Design review of the part built by this model. Coordinates are the model's own, in mm. Face numbers are marked on the shaded views. A direction names the side the tool comes from. Coordinates: 2 decimals unless noted, no trailing zeros. Loops run counter-clockwise (first coordinate to the right, second up) from the corner with the lowest first, then second, coordinate; pieces in that order, holes last. Notation, with made-up numbers: M -3,-15.5 L 22,-15.5 A21 cw 22,2.5 Z; hole C -22.5,87 d3. An arc over 180 degrees is marked long. Write item = value, one per line. Start each with the question number.
from build123d import *

# Parameters (mm, degrees)
EXTRUDE_1_DEPTH       = 15
EXTRUDE_2_DEPTH       = 8
CUT_EXTRUDE_1_DEPTH   = 12
CUT_EXTRUDE_2_DEPTH   = 8
SKETCH_5_R            = 0.5
CUT_EXTRUDE_3_DEPTH   = 317.640652423
SKETCH_6_R            = 2.75
CUT_EXTRUDE_4_DEPTH   = 317.640652423
HOLE_WIZARD_3_0_3_1_D = 6.5
HOLE_WIZARD_M3_1_D    = 2.5


with BuildPart() as part:
    # 草图1 → 凸台-拉伸1 (new body)
    with BuildSketch(Plane.XY):
        with BuildLine():
            Line((154.501486248, 74.365814355), (160.177770707, 76.310041404))
            ThreePointArc((160.177770707, 76.310041404), (169.160526734, 140.718106761), (226.383321785, 171.615364171))
            Line((226.383321785, 171.615364171), (225.315728088, 174.727294301))
            Line((225.315728088, 174.727294301), (234.77220836, 177.96630476))
            Line((234.77220836, 177.96630476), (231.998602564, 186.064008926))
            Line((231.998602564, 186.064008926), (230.57080221, 190.225905867))
            Line((230.57080221, 190.225905867), (233.408459215, 191.199406109))
            Line((233.408459215, 191.199406109), (233.213759167, 191.76693751))
            Line((233.213759167, 191.76693751), (240.591667381, 194.298038138))
            Line((240.591667381, 194.298038138), (240.786367429, 193.730506737))
            Line((240.786367429, 193.730506737), (243.624024434, 194.704006979))
            Line((243.624024434, 194.704006979), (241.482323903, 200.94685239))
            Line((241.482323903, 200.94685239), (129.111106493, 162.396242824))
            Line((129.111106493, 162.396242824), (132.680607379, 151.991500471))
            Line((132.680607379, 151.991500471), (154.501486248, 74.365814355))
        make_face()
    extrude(amount=EXTRUDE_1_DEPTH)

    # 草图2 → 凸台-拉伸2 (add)
    with BuildSketch(Plane(origin=(0, 0, 0), x_dir=(-1, 0, 0), z_dir=(0, 0, -1))):
        Polygon((-174.908927271, 177.441379972), (-194.997272817, 184.33298428), (-193.224414699, 175.267097261), (-181.873786677, 171.373096295), align=None)
    extrude(amount=EXTRUDE_2_DEPTH)

    # 草图3 → 切除-拉伸1 (cut)
    with BuildSketch(Plane.XY.offset(15)):
        with BuildLine():
            Line((148.33581351, 109.973924886), (137.488957816, 148.560574876))
            ThreePointArc((137.488957816, 148.560574876), (137.68708728, 150.700674405), (139.265834382, 152.159042969))
            Line((139.265834382, 152.159042969), (212.284799547, 181.275892717))
            ThreePointArc((212.284799547, 181.275892717), (214.647795853, 181.215617846), (216.233642795, 179.462770427))
            Line((216.233642795, 179.462770427), (217.297595906, 176.361452247))
            ThreePointArc((217.297595906, 176.361452247), (217.048600661, 173.871762608), (214.998888251, 172.436760111))
            ThreePointArc((214.998888251, 172.436760111), (175.157111586, 151.143900213), (155.117593814, 110.657226135))
            ThreePointArc((155.117593814, 110.657226135), (154.455434588, 109.182984766), (153.12452466, 108.266185323))
            Line((153.12452466, 108.266185323), (152.197376559, 107.948113442))
            ThreePointArc((152.197376559, 107.948113442), (149.830188599, 108.129149559), (148.33581351, 109.973924886))
        make_face()
    extrude(amount=-CUT_EXTRUDE_1_DEPTH, mode=Mode.SUBTRACT)

    # 草图4 → 切除-拉伸2 (cut)
    with BuildSketch(Plane.XY.offset(15)):
        Polygon((234.77220836, 177.96630476), (225.315728088, 174.727294301), (222.53974588, 182.819008121), (231.998602564, 186.064008926), align=None)
    extrude(amount=-CUT_EXTRUDE_2_DEPTH, mode=Mode.SUBTRACT)

    # 草图5 → 切除-拉伸3 (cut, through all)
    with BuildSketch(Plane.XY.offset(15)):
        with Locations((228.656571223, 180.394154027)):
            Circle(SKETCH_5_R)
    extrude(amount=-CUT_EXTRUDE_3_DEPTH, mode=Mode.SUBTRACT)

    # 草图6 → 切除-拉伸4 (cut, through all)
    with BuildSketch(Plane.XY.offset(15)):
        with Locations((138.625192324, 159.316929458)):
            Circle(SKETCH_6_R)
        with Locations((222.809016814, 188.197436624)):
            Circle(SKETCH_6_R)
    extrude(amount=-CUT_EXTRUDE_4_DEPTH, mode=Mode.SUBTRACT)

    # Ø3.0 (3) 直径孔1 (through all)
    with Locations(Plane(origin=(-34.303459783, 99.991195485, 0), x_dir=(-0.9458856684292948, -0.32450008052397505, 0), z_dir=(0.32450008052397505, -0.9458856684292948, 0))):
        with Locations((-286.72193914, -5)):
            Hole(HOLE_WIZARD_3_0_3_1_D / 2)

    # M3 螺纹孔1 (through all)
    with Locations(Plane.XY.offset(7)):
        with Locations((228.656571223, 180.394154027)):
            Hole(HOLE_WIZARD_M3_1_D / 2)


solid = part.part
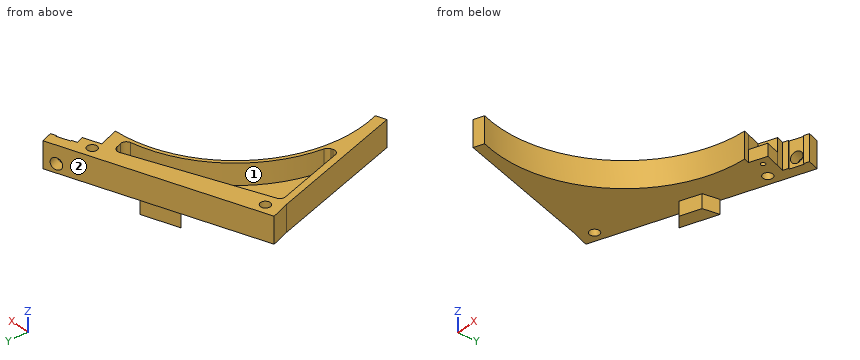
Q1. To check wall thickness, follow line 1 (Y direction, x = 182.5, z = 12.5); line 2 (X direction, y = 134.5, z = 10.5); line 3 (Z direction, x = 149, y = 133). State the ranges of each line that lie inside material, in increasing order. Write a range as from..to.
Q2. Add section B-B on y = 125. State the section outline as (x, z) points, plus the area to 3 significant figures.
Q3. Add section D-D on z = -3. State the section outline as (x, y) points, plus the area to 3 significant figures.
Q4. Add section C-C on x = 205. State the section outline as (y, z) points.
Q5. Clearance check with flat-ended pins moving along their axes: P1, Ø12, axis at x = 204, z = -5, coming from the +Y side; P2, Ø4, axis at y = 152, z = 6, coming from the -X side; P3, Ø2, axis at x = 147.5, z = 11, coming from the +Y side. State where each tip first meets the part, or that it passes through.
Q6. For the marked faces 1 and 2, list the 3-axis set-ups (+Z, -Z, +X, -X, +Y, -Y) from which the entire face can be reached by the end or side of a thin tool; tool diameter is ignored.
Q7. Add section A-A on z = 10.5. State the section outline as (x, y) points.
Values follow:
q1.line_1 = 155.2..157.77, 169.4..180.71
q1.line_2 = 137.6..141.44, 163.02..165.29
q1.line_3 = 0..3
q2.outline = M 140.27,0 L 160.91,0 L 160.91,15 L 158.77,15 L 158.77,3 L 144.11,3 L 144.11,15 L 140.27,15 Z
q2.area = 134 mm2
q3.outline = M 174.91,177.44 L 181.87,171.37 L 193.22,175.27 L 195,184.33 Z
q3.area = 133 mm2
q4.outline = M 167.77,0 L 188.43,0 L 188.43,15 L 178.37,15 L 178.37,3 L 169.88,3 L 169.88,15 L 167.77,15 Z
q5.P1 = 189.23
q5.P2 = 131.99
q5.P3 = 169.05
q6.face_1 = +Z
q6.face_2 = +Z, -Z, -X, +Y
q7.outline = M 129.11,162.4 L 132.68,151.99 L 154.5,74.37 L 160.18,76.31 A72 cw 226.38,171.62 L 222.54,182.82 L 232,186.06 L 230.57,190.23 L 233.41,191.2 L 233.21,191.77 L 240.59,194.3 L 240.79,193.73 L 243.62,194.7 L 241.48,200.95 Z; hole C 138.63,159.32 d5.5; hole M 137.49,148.56 L 148.34,109.97 A3 ccw 152.2,107.95 L 153.12,108.27 A3 ccw 155.12,110.66 A74 cw 215,172.44 A3 ccw 217.3,176.36 L 216.23,179.46 A3 ccw 212.28,181.28 L 139.27,152.16 A3 ccw Z; hole C 222.81,188.2 d5.5
